```python
from build123d import *

# Parameters (mm, degrees)
SKETCH1_W           = 120
SKETCH1_H           = 120
SKETCH1_R           = 36
BOSS_EXTRUDE1_DEPTH = 10


with BuildPart() as part:
    # Sketch1 → Boss-Extrude1 (new body)
    with BuildSketch(Plane(origin=(0, 819.895595987, 0), x_dir=(1, 0, 0), z_dir=(0, 1, 0))):
        with Locations((521.230642584, 440.692981355)):
            Rectangle(SKETCH1_W, SKETCH1_H)
        with Locations(Location((521.230642584, 440.692981355, 0), (0, 0, 90))):
            Circle(SKETCH1_R, mode=Mode.SUBTRACT)
    extrude(amount=-BOSS_EXTRUDE1_DEPTH)


solid = part.part
```
Verification items for the finished model (mm, model axes). Round coordinates to 2 decimals unless told otherwise and drop trailing zeros. Order: outer loops, then holes, each group sorted by start corner. A loop starts at its lowest first (then second) coordinate and runs counter-clockwise, first axis right, second up. Notation, with made-up numbers: (-3, -36) -> (42, -36) arc R28 ccw to (42, 3) -> close; hole circle Ø6 at (-1.75, 36). An arc over 180 degrees is marked (long way). Put each result on its own line as item: value. Start each with the question number.
(1) Section check B-B (z = -406.5). Enter the section's corners in (x, y).
(2) Material ranges on line 1 along X through (y, z) = (817, -468); line 2 along X through (y, z) = (819.75, -466.5); line 3 along Z through (x, y) = (535.5, 819.5), recorded low to high.
(3) Section check A-A (x = 536). Enter the section's corners in (y, z).
(4) Section check C-C (y = 815). Enter the section's corners in (x, z), then the cut area to 3 significant figures.
(5) Draft check along Z on faces 1 (the face through (510.42, 814.97, -475.03)), 2 (the face through (520, 815, -500.693)), 3 (the face through (581.231, 815, -440)). Enter one of: +Z half, -Z half, draft (parallel to the pull), parting line (faces both ways), or undercut.
Completed:
1. outline: (461.23, 809.9) -> (509.97, 809.9) -> (509.97, 819.9) -> (461.23, 819.9) -> close; (532.49, 809.9) -> (581.23, 809.9) -> (581.23, 819.9) -> (532.49, 819.9) -> close
2. line 1: x = 461.23 to 497.77, 544.69 to 581.23
2. line 2: x = 461.23 to 496.13, 546.33 to 581.23
2. line 3: z = -500.69 to -473.74, -407.64 to -380.69
3. outline: (809.9, -500.69) -> (819.9, -500.69) -> (819.9, -473.52) -> (809.9, -473.52) -> close; (809.9, -407.86) -> (819.9, -407.86) -> (819.9, -380.69) -> (809.9, -380.69) -> close
4. outline: (461.23, -500.69) -> (581.23, -500.69) -> (581.23, -380.69) -> (461.23, -380.69) -> close; hole circle Ø72 at (521.23, -440.69)
4. area: 10,300 mm2
5. face 1: undercut
5. face 2: -Z half
5. face 3: draft
